```python
from build123d import *

# Parameters (mm, degrees)
SKETCH1_R           = 66.5
SKETCH1_R_2         = 36.5
BOSS_EXTRUDE1_DEPTH = 320
SKETCH3_R           = 40
CUT_EXTRUDE1_DEPTH  = 79.7
CUT_EXTRUDE2_START  = -31
SKETCH4_R           = 66.5
SKETCH4_R_2         = 64
CUT_EXTRUDE2_DEPTH  = 31
CUT_EXTRUDE3_DEPTH  = 334.533356653


with BuildPart() as part:
    # Sketch1 → Boss-Extrude1 (new body)
    with BuildSketch(Plane.XY):
        Circle(SKETCH1_R)
        Circle(SKETCH1_R_2, mode=Mode.SUBTRACT)
    extrude(amount=BOSS_EXTRUDE1_DEPTH)

    # Sketch3 → Cut-Extrude1 (cut)
    with BuildSketch(Plane.XY.offset(320)):
        Circle(SKETCH3_R)
    cut_extrude1 = extrude(amount=-CUT_EXTRUDE1_DEPTH, mode=Mode.SUBTRACT)

    # Sketch4 → Cut-Extrude2 (cut)
    with BuildSketch(Plane.XY.offset(320).offset(CUT_EXTRUDE2_START)):
        Circle(SKETCH4_R)
        Circle(SKETCH4_R_2, mode=Mode.SUBTRACT)
    cut_extrude2 = extrude(amount=CUT_EXTRUDE2_DEPTH, mode=Mode.SUBTRACT)

    # Mirror1: Cut-Extrude1, Cut-Extrude2 across plane
    add(cut_extrude1.mirror(Plane.XY.offset(160)), mode=Mode.SUBTRACT)
    add(cut_extrude2.mirror(Plane.XY.offset(160)), mode=Mode.SUBTRACT)

    # Sketch5 → Cut-Extrude3 (cut, through all)
    with BuildSketch(Plane.XY.offset(320)):
        with BuildLine():
            Line((64.899922958, 14.5), (53.899922958, 14.5))
            Line((53.899922958, 14.5), (44.558079818, 49.364233235))
            ThreePointArc((44.558079818, 49.364233235), (57.43816051, 33.512799305), (64.899922958, 14.5))
        make_face()
    extrude(amount=-CUT_EXTRUDE3_DEPTH, mode=Mode.SUBTRACT)


solid = part.part
```
Verification items for the finished model (mm, model axes). A direction names the side the tool comes from. Give positions to 0.01 mm unless a question says otherwise; leave off trailing zeros. Order: outer loops, then holes, each group sorted by start corner. A loop starts at its lowest first (then second) coordinate and runs counter-clockwise, first axis right, second up. Notation, with made-up numbers: M 32.25,76 L 57.25,76 A26 cw 57.25,90 Z; hole C 28.25,86.25 d11. An arc over 180 degrees is marked long. Return JSON: item names as keys, results as strings. Group by question number.
1) Section check A-A on x = 0. Record the cut outline in (y, z), and give its area (3 significant figures).
2) Scan lines: line 1 (Y direction, x = 0, z = 144); line 2 (Y direction, x = 0, z = 274). Record each from-to range of solid material in increasing order.
3) Mould release check, pull along Y, two halves, no side actions. Record for faces 1 (the face through (-59.4, 24.9, 289)), 2 (the face through (-8.67, -39.05, 39.29)), 3 (the face through (-7.912, -35.632, 158.876)), 4 (the face through (-58.72, -31.21, 158.19)): pulls with the +Y half, pulls with the -Y half, needs draft (parallel to the pull), parting line crosses it, or undercut.
4) Access from +Z, -Z, +X, -X, +Y, -Y to the whole of each face (thin tool, end or side, straight path). Record for faces 5 (the face through (-57.33, -28.45, 304.28)), 6 (the face through (-59.4, 24.9, 31)), 7 (the face through (59, 14.5, 162)).
5) Section check C-C on z = 237. Record the cut outline in (x, y), and give its area (3 significant figures).
6) Go/stop test with flat-tipped pins: pin 1 Ø12 at (x, z) = (-13.5, 41) entering from -Y; pin 2 Ø2 at (y, z) = (-39, 221.5) entering from -X; pin 3 Ø6 at (y, z) = (-52.5, 57) entering from +X; pin 4 Ø24 at (x, y) = (-8.5, 11) entering from +Z. Record where each tip stops, or that it passes through.
7) Section check D-D on x = -49.5. Record the cut outline in (y, z), and give its area (3 significant figures).
Answer block:
{
 "1": {"outline": "M -66.5,31 L -64,31 L -64,0 L -40,0 L -40,79.7 L -36.5,79.7 L -36.5,240.3 L -40,240.3 L -40,320 L -64,320 L -64,289 L -66.5,289 Z; M 36.5,79.7 L 40,79.7 L 40,0 L 64,0 L 64,31 L 66.5,31 L 66.5,289 L 64,289 L 64,320 L 40,320 L 40,240.3 L 36.5,240.3 Z", "area": "17,800 mm^2"},
 "2": {"line 1": "y = -66.5 to -36.5, 36.5 to 66.5", "line 2": "y = -66.5 to -40, 40 to 66.5"},
 "3": {"face 1": "needs draft", "face 2": "undercut", "face 3": "undercut", "face 4": "parting line crosses it"},
 "4": {"face 5": "+Z", "face 6": "-Z", "face 7": "+Z, -Z, +X, +Y"},
 "5": {"outline": "M 44.56,49.36 A66.5 ccw long 64.9,14.5 L 53.9,14.5 Z; hole C 0,0 d73", "area": "9,430 mm^2"},
 "6": {"pin 1": "stops at y = -66.08", "pin 2": "stops at x = -54.57", "pin 3": "stops at x = 44.41", "pin 4": "passes through"},
 "7": {"outline": "M -44.41,31 L -40.57,31 L -40.57,0 L 40.57,0 L 40.57,31 L 44.41,31 L 44.41,289 L 40.57,289 L 40.57,320 L -40.57,320 L -40.57,289 L -44.41,289 Z", "area": "27,900 mm^2"}
}
